For this review, take the finished solid that the model builds, in its own axes (mm). A direction names the side the tool comes from. Give positions to 0.01 mm unless a question says otherwise; leave off trailing zeros. Loops run counter-clockwise (first coordinate to the right, second up) from the corner with the lowest first, then second, coordinate; pieces in that order, holes last. Notation, with made-up numbers: (38.5, -17) -> (54.5, -17) arc R27 cw to (54.5, 21) -> close; hole circle Ø5 at (28, -9). An arc over 180 degrees is marked (long way). Write each question's results on one line, items separated by ' | '. Start each with the question number.
```python
from build123d import *

# Parameters (mm, degrees)
BASE_BLOCK_DEPTH = 11
TOP_PLATE_DEPTH  = 12
GUSSET_RIB_DEPTH = 11
CUT_22_PROFILE_R = 11
CUT_22_DEPTH     = 11


with BuildPart() as part:
    # Base Block Profile → Base Block (new body)
    with BuildSketch(Plane.XY):
        with BuildLine():
            Line((58, 0), (58, -52))
            Line((58, -52), (18, -52))
            ThreePointArc((18, -52), (5.272077939, -46.727922061), (0, -34))
            Line((0, -34), (0, 0))
            Line((0, 0), (58, 0))
        make_face()
    extrude(amount=BASE_BLOCK_DEPTH)

    # Top Plate Profile → Top Plate (add)
    with BuildSketch(Plane(origin=(0, 0, 0), x_dir=(1, 0, 0), z_dir=(0, 1, 0))):
        Polygon((58, -11), (58, -39), (37, -39), (37, -31), (23, -31), (23, -39), (15, -39), (15, -18), (0, -18), (0, -11), align=None)
    extrude(amount=-TOP_PLATE_DEPTH)

    # Gusset Profile → Gusset Rib (add)
    with BuildSketch(Plane(origin=(58, 0, 0), x_dir=(0, 0, -1), z_dir=(1, 0, 0))):
        Polygon((-11, -12), (-31, -12), (-11, -43), align=None)
    extrude(amount=-GUSSET_RIB_DEPTH)

    # Cut Ø22 Profile → Cut Ø22 (cut)
    with BuildSketch(Plane.XY.offset(11)):
        with Locations((18, -34)):
            Circle(CUT_22_PROFILE_R)
    extrude(amount=-CUT_22_DEPTH, mode=Mode.SUBTRACT)


solid = part.part
```
1. We need section A-A (y = -37). Write out the cut boundary in (x, z).
2. Wall thickness on L1, parallel to Y at x = 18, z = 4; L2, parallel to Z at x = 8.5, y = -13.5; L3, parallel to X at y = -32.5, z = 16: over which ranges is each line inside the solid? List them lowest first.
3. We need section B-B (x = 35). Write out the cut boundary in (y, z), plus the area to 3 significant figures.
4. Draft analysis for pull direction X (two halves, no side actions). For faces 1 (the flat face through (23, -6, 35)), 2 (the flat face through (0, -13, 7)), 3 (the flat face through (29, -26, 0)), state which applies: released by +X, released by -X, zero draft, split by the parting line, or undercut.
5. We need section C-C (z = 8.5). Write out the cut boundary in (x, y), plus the area to 3 significant figures.
6. We need section D-D (z = 16). Write out the cut boundary in (x, y), plus the area to 3 significant figures.
7. Machinability: for faces 4 (the flat face through (47, -20, 17)), 5 (the flat face through (37, -6, 35)), 6 (the flat face through (15, -6, 29)), which of the approach directions +Z, -Z, +X, -X, +Y, -Y give a long, thin tool a straight path to every point of the face, cutting with its end or side? Answer none if there is none.
8. For pin 1 Ø3.5 at (y, z) = (-3, 29.5) entering from -X; pin 2 Ø10 at (x, y) = (27, -25.5) entering from +Z; pin 3 Ø3.5 at (x, y) = (33.5, -5) entering from +Z, all flat-tipped, find the tip position at first contact; note any pin that passes through.
Response:
1) outline: (0.25, 0) -> (7.42, 0) -> (7.42, 11) -> (0.25, 11) -> close; (28.58, 0) -> (58, 0) -> (58, 14.87) -> (47, 14.87) -> (47, 11) -> (28.58, 11) -> close
2) L1: y = -52 to -45, -23 to 0 | L2: z = 0 to 11 | L3: x = 47 to 58
3) outline: (-52, 0) -> (0, 0) -> (0, 31) -> (-12, 31) -> (-12, 11) -> (-52, 11) -> close | area: 812 mm2
4) face 1: undercut | face 2: released by -X | face 3: zero draft
5) outline: (0, -34) arc R18 ccw to (18, -52) -> (58, -52) -> (58, 0) -> (0, 0) -> close; hole circle Ø22 at (18, -34) | area: 2,570 mm2
6) outline: (0, -12) -> (47, -12) -> (47, -35.25) -> (58, -35.25) -> (58, 0) -> (0, 0) -> close | area: 952 mm2
7) face 4: +Z, -X, -Y | face 5: +Z, +Y, -Y | face 6: +Z, -X, +Y, -Y
8) pin 1: stops at x = 15 | pin 2: stops at z = 11 | pin 3: stops at z = 31
